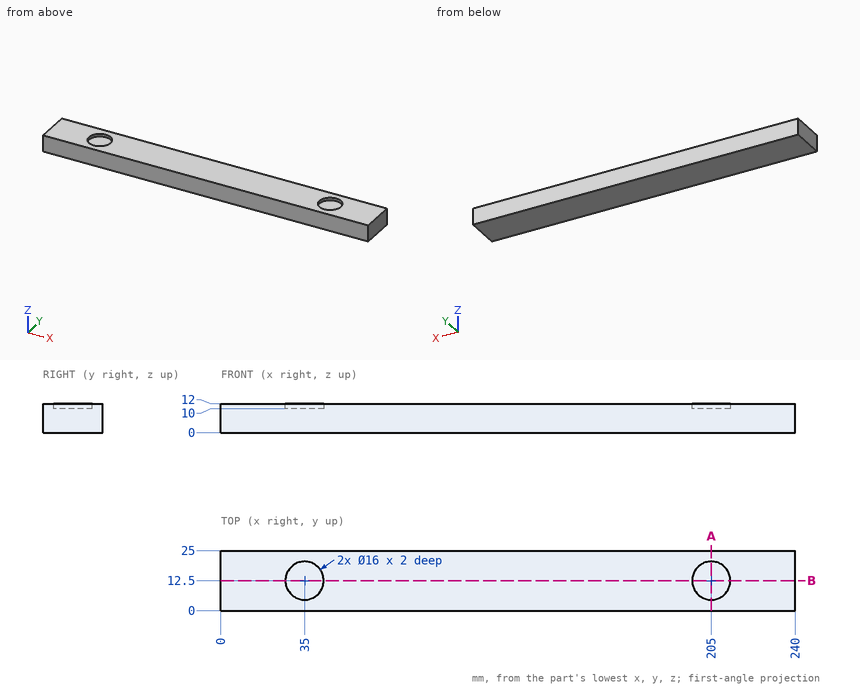
The figure shows three views and two pictorial views of one solid part (mm, origin at its lowest corner). Answer the questions. Coordinates: 2 decimals unless noted, no trailing zeros. Loops run counter-clockwise (first coordinate to the right, second up) from the corner with the lowest first, then second, coordinate; pieces in that order, holes last. Notation, with made-up numbers: M 8,28 L 31,28 A18 ccw 31,61 Z; hole C 20,-37.5 d9. An arc over 180 degrees is marked long. Answer as CSV lines item,"result". Start each with the question number.
(1) Find the intervals of material crossed by L1, parallel to Y at x = 35, z = 10.65; L2, parallel to X at y = 7.5, z = 11.5 (3 decimals); L3, parallel to X at y = 15.75, z = 10.25, in increasing order. Write a range as [from, to].
(2) The part is cut by section A-A (x = 205). Give the vertices of the cut face in (y, z), and give its area (3 significant figures).
(3) The part is cut by section B-B (y = 12.5). Give the vertices of the cut face in (x, z), and give its area (3 significant figures).
(4) Given pin 1 (8 mm diameter, centred on x = 38.5, y = 11, fed in from +Z), flat-ended and moving along its own axis, determine where the tip first touches the part or whether it passes through.
Determined:
1,L1,"[0, 4.5], [20.5, 25]"
1,L2,"[0, 28.755], [41.245, 198.755], [211.245, 240]"
1,L3,"[0, 27.69], [42.31, 197.69], [212.31, 240]"
2,outline,"M 0,0 L 25,0 L 25,12 L 20.5,12 L 20.5,10 L 4.5,10 L 4.5,12 L 0,12 Z"
2,area,"268 mm2"
3,outline,"M 0,0 L 240,0 L 240,12 L 213,12 L 213,10 L 197,10 L 197,12 L 43,12 L 43,10 L 27,10 L 27,12 L 0,12 Z"
3,area,"2,820 mm2"
4,pin 1,"z = 10"
